from build123d import *

# Parameters (mm, degrees)
SKETCH_1_R      = 2.1
EXTRUDE_1_DEPTH = 3


with BuildPart() as part:
    # 草图1 → 凸台-拉伸1 (new body)
    with BuildSketch(Plane(origin=(0, 0, 0), x_dir=(1, 0, 0), z_dir=(0, 1, 0))):
        with BuildLine():
            Line((-17, -15), (17, -15))
            ThreePointArc((17, -15), (19.121320344, -14.121320344), (20, -12))
            Line((20, -12), (20, 12))
            ThreePointArc((20, 12), (19.121320344, 14.121320344), (17, 15))
            Line((17, 15), (-17, 15))
            ThreePointArc((-17, 15), (-19.121320344, 14.121320344), (-20, 12))
            Line((-20, 12), (-20, -12))
            ThreePointArc((-20, -12), (-19.121320344, -14.121320344), (-17, -15))
        make_face()
        with Locations(Location((-15, 10, 0), (0, 0, 270))):
            Circle(SKETCH_1_R, mode=Mode.SUBTRACT)
        with Locations(Location((15, 10, 0), (0, 0, 270))):
            Circle(SKETCH_1_R, mode=Mode.SUBTRACT)
        with Locations(Location((-15, -10, 0), (0, 0, 270))):
            Circle(SKETCH_1_R, mode=Mode.SUBTRACT)
        with Locations(Location((15, -10, 0), (0, 0, 270))):
            Circle(SKETCH_1_R, mode=Mode.SUBTRACT)
        with BuildLine():
            Line((-9, -8), (9, -8))
            ThreePointArc((9, -8), (11.121320344, -7.121320344), (12, -5))
            Line((12, -5), (12, 5))
            ThreePointArc((12, 5), (11.121320344, 7.121320344), (9, 8))
            Line((9, 8), (-9, 8))
            ThreePointArc((-9, 8), (-11.121320344, 7.121320344), (-12, 5))
            Line((-12, 5), (-12, -5))
            ThreePointArc((-12, -5), (-11.121320344, -7.121320344), (-9, -8))
        make_face(mode=Mode.SUBTRACT)
    extrude(amount=EXTRUDE_1_DEPTH)


solid = part.part
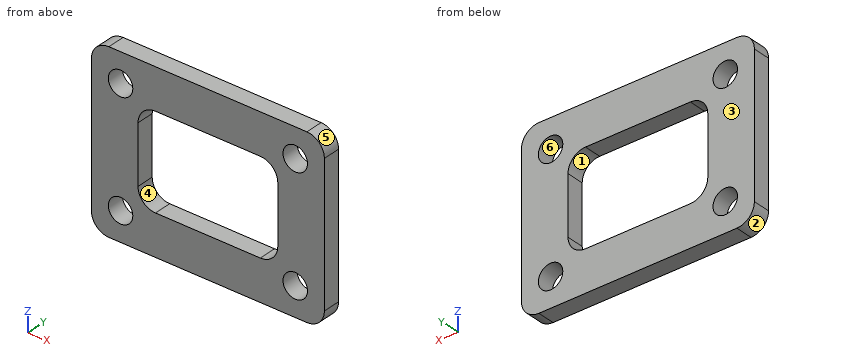
Input: part model. Units: mm. Frame: model coordinates. Face numbers are marked on the shaded views. A direction names the side the tool comes from. Give positions to 0.01 mm unless a question says otherwise; leave off trailing zeros. Loops run counter-clockwise (first coordinate to the right, second up) from the corner with the lowest first, then second, coordinate; pieces in that order, holes last. Notation, with made-up numbers: M 45.5,5 L 90.5,5 A9 cw 90.5,17 Z; hole C 66.5,27.5 d6. An arc over 180 degrees is marked long. Use one line per item in the form item = value.
1. Section query C-C, the plane y = 0.5. Return the cut outline in (x, z), and give its area (3 significant figures).
Numbers:
outline = M -20,-12 A3 ccw -17,-15 L 17,-15 A3 ccw 20,-12 L 20,12 A3 ccw 17,15 L -17,15 A3 ccw -20,12 Z; hole C -15,-10 d4.2; hole C -15,10 d4.2; hole M -12,-5 A3 ccw -9,-8 L 9,-8 A3 ccw 12,-5 L 12,5 A3 ccw 9,8 L -9,8 A3 ccw -12,5 Z; hole C 15,-10 d4.2; hole C 15,10 d4.2
area = 761 mm²
2. Section query A-A, the plane x = 7.5. Return the cut outline in (y, z).
Numbers:
outline = M 0,-15 L 3,-15 L 3,-8 L 0,-8 Z; M 0,8 L 3,8 L 3,15 L 0,15 Z
3. Section query D-D, the plane x = -15. Return the cut outline in (y, z), and give its area (3 significant figures).
Numbers:
outline = M 0,-15 L 3,-15 L 3,-12.1 L 0,-12.1 Z; M 0,-7.9 L 3,-7.9 L 3,7.9 L 0,7.9 Z; M 0,12.1 L 3,12.1 L 3,15 L 0,15 Z
area = 64.8 mm²
4. Line query: L1, parallel to X at y = 1.1, z = -10; L2, parallel to X at y = 1.9, z = 9.5; L3, parallel to X at y = 0.5, z = -2.5. Output: solid intervals per line, ascending.
Numbers:
L1 = -20 to -17.1, -12.9 to 12.9, 17.1 to 20
L2 = -20 to -17.04, -12.96 to 12.96, 17.04 to 20
L3 = -20 to -12, 12 to 20
5. First-contact query: pin 1 (1.5 mm diameter, centred on x = 11.5, z = -8, fed in from -Y). Flat tip, straight axial feed; report the tip coordinate or a pass-through.
Numbers:
pin_1 = 0
6. Section query B-B, the plane z = -10. Return the cut outline in (x, y).
Numbers:
outline = M -20,0 L -17.1,0 L -17.1,3 L -20,3 Z; M -12.9,0 L 12.9,0 L 12.9,3 L -12.9,3 Z; M 17.1,0 L 20,0 L 20,3 L 17.1,3 Z
7. Pull-direction query (Z, two-part tool) for the marked faces 3, 4, 5 and 6; classes: released by +Z, released by -Z, zero draft, split by the parting line, or undercut.
Numbers:
face_3 = zero draft
face_4 = undercut
face_5 = released by +Z
face_6 = undercut
8. Reachability of the marked faces 1 and 2 from +Z, -Z, +X, -X, +Y, -Y: full face, straight path, thin tool, end or side. Return the list, or none.
Numbers:
face_1 = +Y, -Y
face_2 = -Z, -X, +Y, -Y
